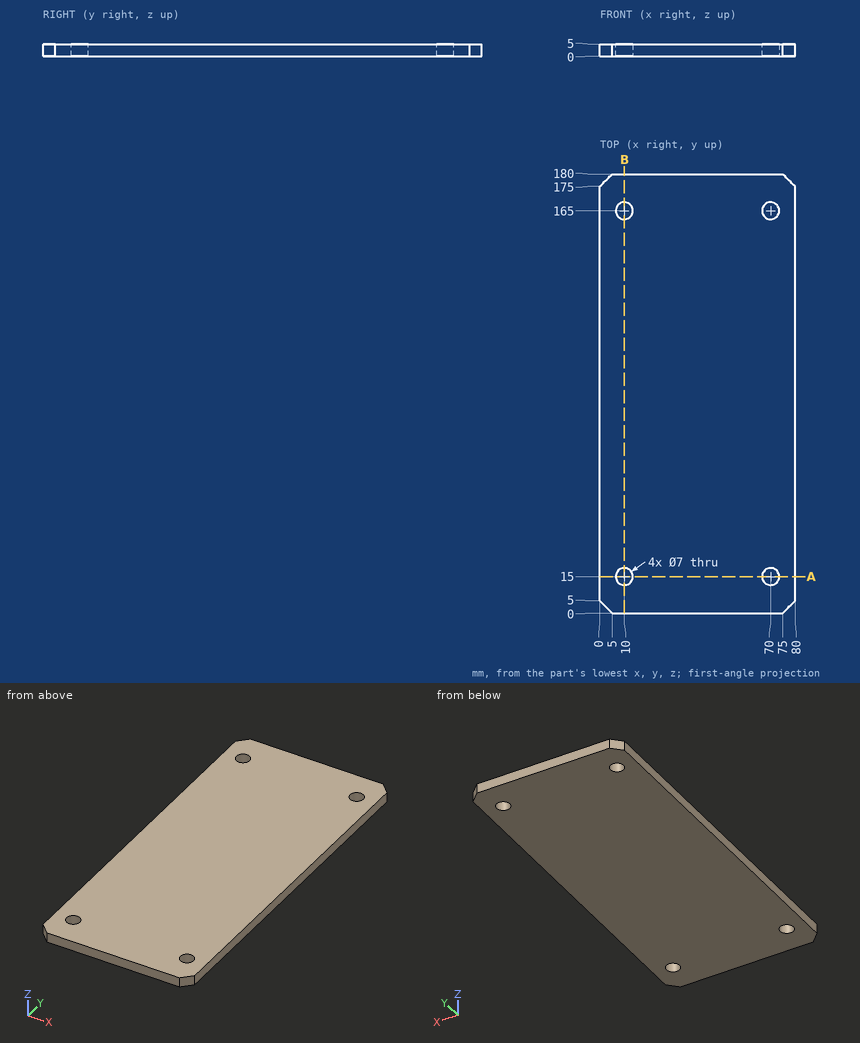
Drawing for the job (mm, zero at the part's lowest x, y, z). Round coordinates to 2 decimals unless told otherwise and drop trailing zeros. Order: outer loops, then holes, each group sorted by start corner. A loop starts at its lowest first (then second) coordinate and runs counter-clockwise, first axis right, second up. Notation, with made-up numbers: (-26.75, 40) -> (22.25, 40) arc R31 cw to (22.25, 72) -> close; hole circle Ø7 at (-1.75, -21.75). An arc over 180 degrees is marked (long way). Put each result on its own line as item: value.
Q1. Band-saw the part on A-A (y = 15). Give the cut face in (x, z), and give its area (3 significant figures).
From the geometry:
outline: (0, 0) -> (6.5, 0) -> (6.5, 5) -> (0, 5) -> close; (13.5, 0) -> (66.5, 0) -> (66.5, 5) -> (13.5, 5) -> close; (73.5, 0) -> (80, 0) -> (80, 5) -> (73.5, 5) -> close
area: 330 mm2
Q2. Band-saw the part on B-B (x = 10). Give the cut face in (y, z).
From the geometry:
outline: (0, 0) -> (11.5, 0) -> (11.5, 5) -> (0, 5) -> close; (18.5, 0) -> (161.5, 0) -> (161.5, 5) -> (18.5, 5) -> close; (168.5, 0) -> (180, 0) -> (180, 5) -> (168.5, 5) -> close
Q3. Wall check: line 1 (Y direction, x = 10, z = 3.2); line 2 (X direction, y = 165, z = 3.2); line 3 (Y direction, x = 67, z = 0.95). Give the ranges that are in metal, low to high. Write a range as [from, to].
From the geometry:
line 1: y = [0, 11.5], [18.5, 161.5], [168.5, 180]
line 2: x = [0, 6.5], [13.5, 66.5], [73.5, 80]
line 3: y = [0, 13.2], [16.8, 163.2], [166.8, 180]
